Answer from the drawing. Dimensions are ordinates in mm from the lowest x, y and z of the part. A direction names the side the tool comes from. Round coordinates to 2 decimals unless told otherwise and drop trailing zeros. Write each loop counter-clockwise with the first axis right and the second up, starting at its lowest first coordinate (ties: lowest second). Pieces come first, ordered by that corner, then holes. Notation, with made-up numbers: (7.25, 74) - (53.25, 74) arc R22 ccw to (53.25, 105) - close; hole circle Ø5 at (68.25, 53.5). An arc over 180 degrees is marked (long way). One line per item, written item: value. Start each with the question number.
(1) Flat-ended cylindrical pins translate along their axes: pin 1 Ø9 at (y, z) = (5.8, 5.8) entering from +X; pin 2 Ø12 at (x, y) = (21, 33) entering from -Z; pin 3 Ø6 at (x, y) = (18, 6.5) entering from -Z. Find the tip coordinate at first contact, or state that the pin passes through.
(2) The mould has two halves that part along Z. Classify the marked faces 3, 4, 5 and 6: +Z half, -Z half, draft (parallel to the pull), parting line (faces both ways), or undercut.
(3) For the marked faces 1 and 2, determine the directions among +Z, -Z, +X, -X, +Y, -Y from which every point of the face is accessible in a straight line to the end or side of a thin tool.
(4) A cutting plane is placed at C-C, the plane y = 7.5. Determine the outline of the cut face in (x, z), plus the area to 3 significant figures.
(5) A cutting plane is placed at A-A, the plane y = 21. Determine the outline of the cut face in (x, z).
(6) Find the intervals of material crossed by L1, parallel to Z at x = 3, y = 5.5; L2, parallel to Y at x = 19.5, z = 21; L3, parallel to X at y = 5, z = 8.5, in increasing order.
(7) A cutting plane is placed at D-D, the plane x = 24.5. Determine the outline of the cut face in (y, z).
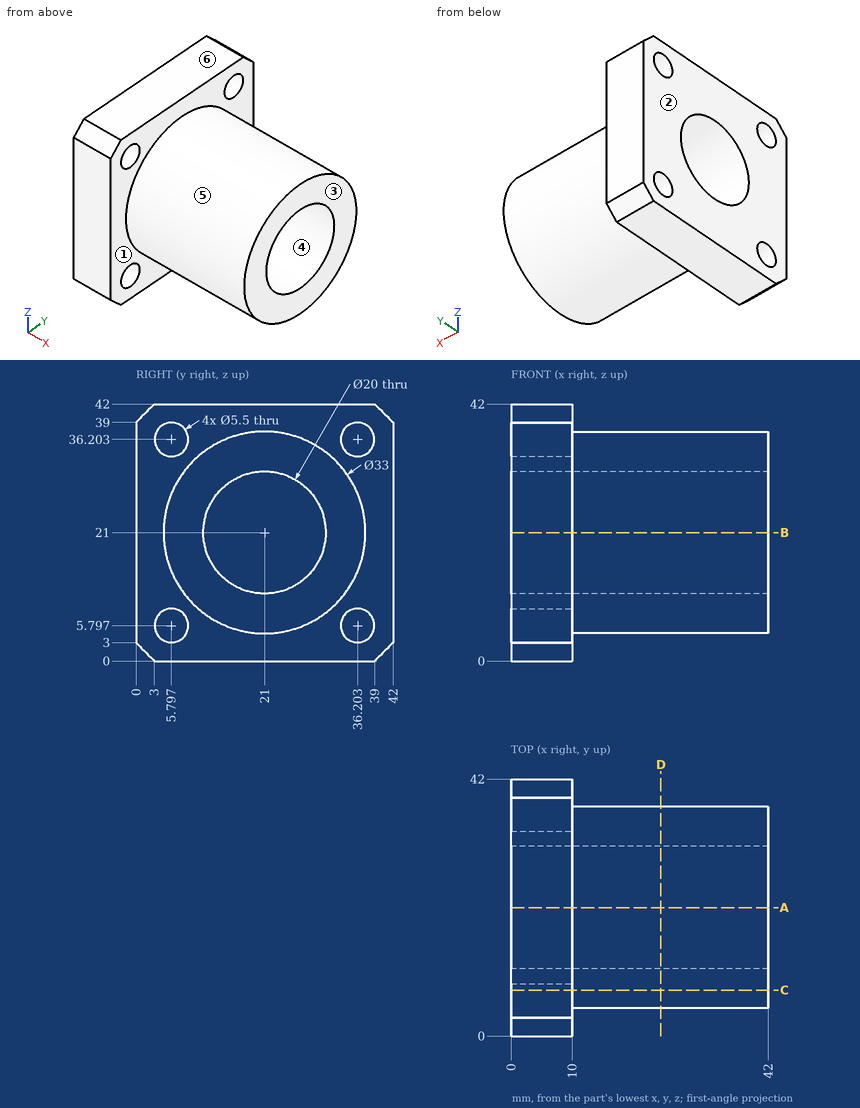
Here are the results:
1. pin 1: x = 10
1. pin 2: z = 5.63
1. pin 3: z = 9.17
2. face 3: draft
2. face 4: undercut
2. face 5: parting line
2. face 6: +Z half
3. face 1: +X
3. face 2: +Z, -Z, -X, +Y, -Y
4. outline: (0, 0) - (10, 0) - (10, 3.64) - (0, 3.64) - close; (0, 7.96) - (10, 7.96) - (10, 11.51) - (42, 11.51) - (42, 30.49) - (10, 30.49) - (10, 34.04) - (0, 34.04) - close; (0, 38.36) - (10, 38.36) - (10, 42) - (0, 42) - close
4. area: 941 mm²
5. outline: (0, 0) - (10, 0) - (10, 4.5) - (42, 4.5) - (42, 11) - (0, 11) - close; (0, 31) - (42, 31) - (42, 37.5) - (10, 37.5) - (10, 42) - (0, 42) - close
6. L1: 0 to 3.06, 8.53 to 33.47, 38.94 to 42
6. L2: 4.5 to 11, 31 to 37.5
6. L3: 0 to 10
7. outline: circle Ø33 at (21, 21); hole circle Ø20 at (21, 21)
